Job drawing, mm, ordinate dimensions from the low corner. One solid piece. Coordinates: 2 decimals unless noted, no trailing zeros. Order: outer loops, then holes, each group sorted by start corner. A loop starts at its lowest first (then second) coordinate and runs counter-clockwise, first axis right, second up. Notation, with made-up numbers: (-18, 10.25) - (1, 10.25) arc R25 ccw to (1, 23.25) - close; hole circle Ø4 at (36.5, 47). An arc over 180 degrees is marked (long way). Use one line per item in the form item = value.
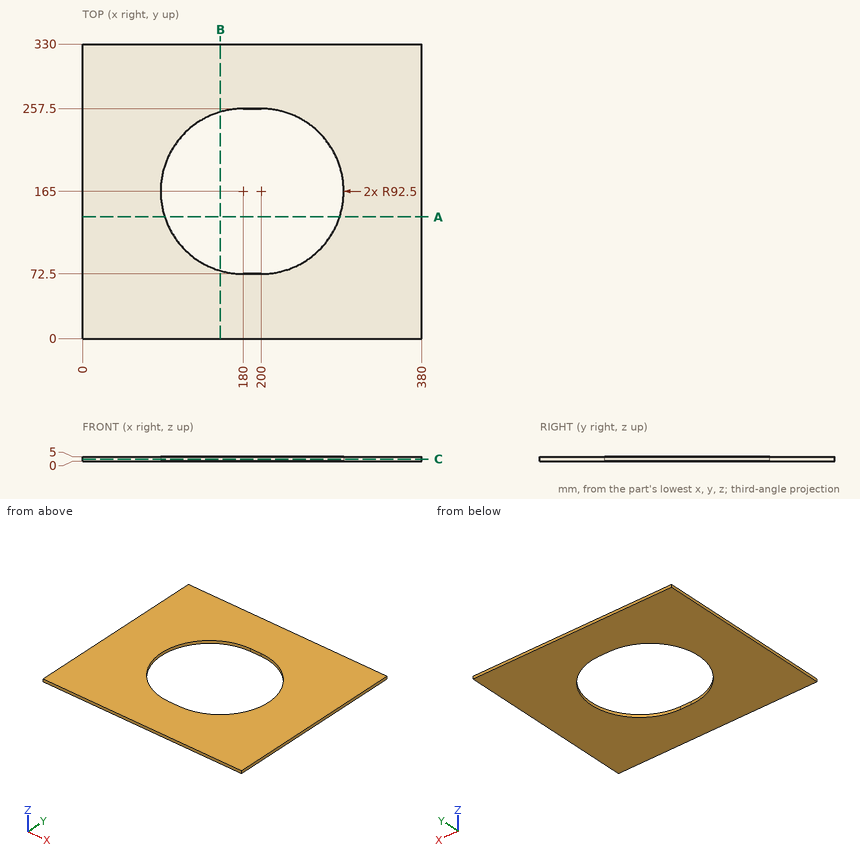
Item 1: Drill centre lines: line 1 (X direction, y = 202, z = 4.85); line 2 (X direction, y = 222.5, z = 4.55); line 3 (Y direction, x = 160, z = 2.8). Where is each one in solid material? Low to high. Write a range as [from, to].
Derived:
line_1 = [0, 95.22], [284.78, 380]
line_2 = [0, 107.54], [272.46, 380]
line_3 = [0, 74.69], [255.31, 330]
Item 2: Cut at A-A, the plane y = 136.5. Write the cut outline in (x, z).
Derived:
outline = (0, 0) - (92, 0) - (92, 5) - (0, 5) - close; (288, 0) - (380, 0) - (380, 5) - (288, 5) - close
Item 3: Cut at C-C, the plane z = 2.3. Write the cut outline in (x, y), plus the area to 3 significant figures.
Derived:
outline = (0, 0) - (380, 0) - (380, 330) - (0, 330) - close; hole (180, 72.5) - (200, 72.5) arc R92.5 ccw to (200, 257.5) - (180, 257.5) arc R92.5 ccw to start
area = 94,800 mm²
Item 4: Cut at B-B, the plane x = 154.5. Write the cut outline in (y, z).
Derived:
outline = (0, 0) - (76.08, 0) - (76.08, 5) - (0, 5) - close; (253.92, 0) - (330, 0) - (330, 5) - (253.92, 5) - close
